```python
from build123d import *

# Parameters (mm, degrees)
SKETCH_1_W      = 30
SKETCH_1_H      = 60
SKETCH_1_W_2    = 24
SKETCH_1_H_2    = 54
EXTRUDE_1_DEPTH = 100


with BuildPart() as part:
    # 草图1 → 拉伸-薄壁1 (new body)
    with BuildSketch(Plane.XY):
        Rectangle(SKETCH_1_W, SKETCH_1_H)
        Rectangle(SKETCH_1_W_2, SKETCH_1_H_2, mode=Mode.SUBTRACT)
    extrude(amount=EXTRUDE_1_DEPTH)


solid = part.part
```
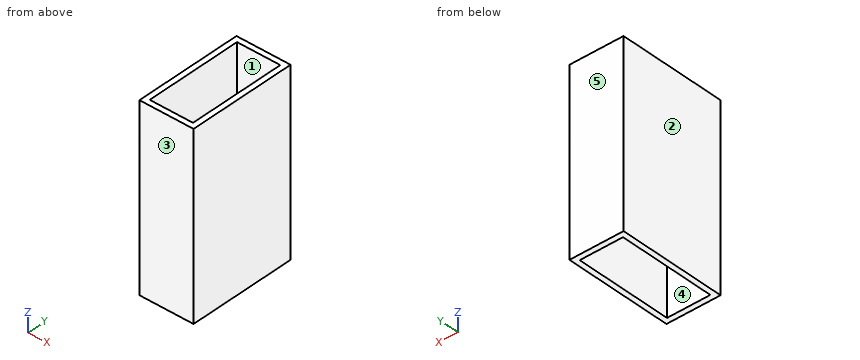
Could you check a few things on this model? Use its own coordinates, in mm. Face numbers are marked on the shaded views. A direction names the side the tool comes from. Give positions to 0.01 mm unless a question says otherwise; leave off trailing zeros. Loops run counter-clockwise (first coordinate to the right, second up) from the corner with the lowest first, then second, coordinate; pieces in that order, holes last. Notation, with made-up numbers: (3.5, 9.5) - (37.5, 9.5) arc R20 ccw to (37.5, 40.5) - close; hole circle Ø5 at (-5, 70.25). An arc over 180 degrees is marked (long way). Answer in a Markdown table with one row per item. Add a question column.
Q1. For pin 1 (8 mm diameter, centred on x = -6.5, y = -19.5, fed in from +Z), with a flat end and sliding along its axis, tell me the tip position at first contact or that it passes through.
Q2. Which directions (+Z, -Z, +X, -X, +Y, -Y) give clear straight access to the entire face, cutting with the end or side of a thin tool? Please do the marked faces 1 and 2.
Q3. If we section it at C-C (y = -15.5): List the corners of the cut face in (x, z) for me.
Q4. If we section it at A-A (x = -6): List the corners of the cut face in (y, z) for me.
Q5. If we section it at B-B (z = 32): List the corners of the cut face in (x, y) for me, plus the area to 3 significant figures.
Q6. We'd pull the mould along Y, two halves only. Please class the marked faces 3, 4 and 5: +Y half, -Y half, draft (parallel to the pull), parting line (faces both ways), or undercut.
Q7. Please list where these lines run through material, in increasing order: L1, parallel to X at y = -21, z = 89; L2, parallel to Y at x = 0.5, z = 71.5. Write a range as from..to.
The answers:
| question | item | result |
|---|---|---|
| 1 | pin 1 | passes through |
| 2 | face 1 | +Z, -Z |
| 2 | face 2 | +Z, -Z, -X, +Y, -Y |
| 3 | outline | (-15, 0) - (-12, 0) - (-12, 100) - (-15, 100) - close; (12, 0) - (15, 0) - (15, 100) - (12, 100) - close |
| 4 | outline | (-30, 0) - (-27, 0) - (-27, 100) - (-30, 100) - close; (27, 0) - (30, 0) - (30, 100) - (27, 100) - close |
| 5 | outline | (-15, -30) - (15, -30) - (15, 30) - (-15, 30) - close; hole (-12, -27) - (12, -27) - (12, 27) - (-12, 27) - close |
| 5 | area | 504 mm^2 |
| 6 | face 3 | -Y half |
| 6 | face 4 | undercut |
| 6 | face 5 | +Y half |
| 7 | L1 | x = -15..-12, 12..15 |
| 7 | L2 | y = -30..-27, 27..30 |
